Geometry: see drawing. Coordinates: mm, zero at the bounding-box minimum. A direction names the side the tool comes from. Round coordinates to 2 decimals unless told otherwise and drop trailing zeros. Loops run counter-clockwise (first coordinate to the right, second up) from the corner with the lowest first, then second, coordinate; pieces in that order, holes last. Notation, with made-up numbers: (45, 36.25) - (94, 36.25) arc R14 ccw to (94, 47.25) - close; hole circle Ø11 at (31.5, -27.5). An arc over 180 degrees is marked (long way). Return JSON: item names as keys, results as strings. Group by question number.
1. Material intervals for probe 1 along Y at (x, z) = (62.5, 27.5); probe 2 along Z at (x, y) = (254.5, 7.5), sorted ascending.
2. Section A-A on x = 172. Return loops of the section in (y, z), and give its area (3 significant figures).
3. Set-up query: the marked faces 1 and 2. Return all of +Z, -Z, +X, -X, +Y, -Y with unobstructed straight access to the full face (end or side cutting, diameter ignored); none if empty.
4. First-contact query: pin 1 Ø1.5 at (x, z) = (179.5, 38) entering from +Y; pin 2 Ø10 at (x, z) = (120.5, 23.5) entering from -Y. Flat tips, straight axial feed; report the tip coordinate or a pass-through.
5. Section B-B on y = 64.5. Return loops of the section in (x, z), and give its area (3 significant figures).
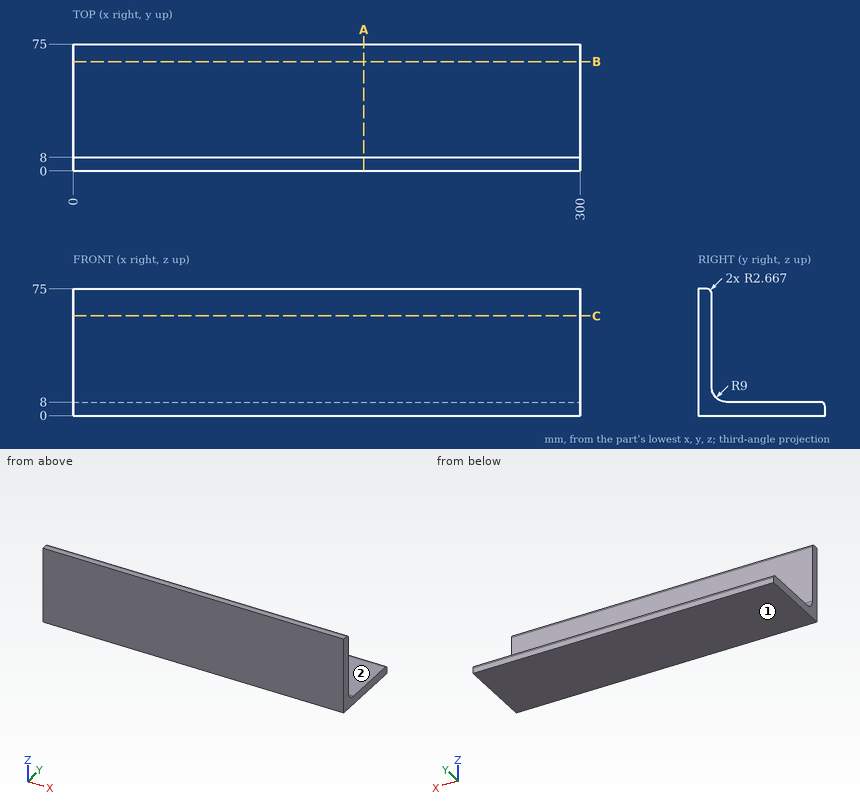
Taken from the geometry:
{
 "1": {"probe 1": "0 to 8", "probe 2": "0 to 73.89"},
 "2": {"outline": "(0, 0) - (75, 0) - (75, 5.33) arc R2.67 ccw to (72.33, 8) - (17, 8) arc R9 cw to (8, 17) - (8, 72.33) arc R2.67 ccw to (5.33, 75) - (0, 75) - close", "area": "1,150 mm2"},
 "3": {"face 1": "-Z, +X, -X, +Y, -Y", "face 2": "+Z, +X, -X, +Y"},
 "4": {"pin 1": "y = 8", "pin 2": "y = 0"},
 "5": {"outline": "(0, 0) - (300, 0) - (300, 8) - (0, 8) - close", "area": "2,400 mm2"}
}
